The figure shows three views and two pictorial views of one solid part (mm, origin at its lowest corner). Answer the questions. A direction names the side the tool comes from. Coordinates: 2 decimals unless noted, no trailing zeros. Order: outer loops, then holes, each group sorted by start corner. A loop starts at its lowest first (then second) coordinate and runs counter-clockwise, first axis right, second up. Notation, with made-up numbers: (88.25, -30.75) -> (115.25, -30.75) arc R18 ccw to (115.25, -9.75) -> close; hole circle Ø3 at (2, 27). An arc over 180 degrees is marked (long way). Write item = value, one per line.
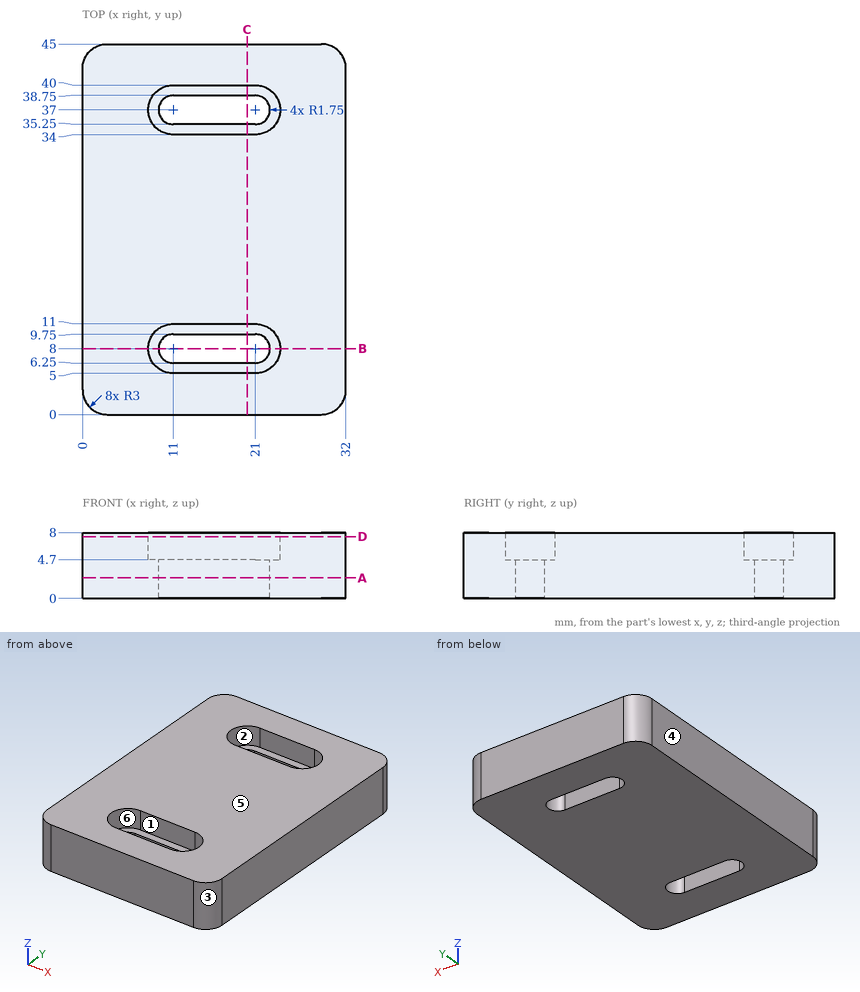
Q1. Section B-B, the plane y = 8 is taken. Give the vertices of the cut face in (x, z).
The answers:
outline = (0, 0) -> (9.25, 0) -> (9.25, 4.7) -> (8, 4.7) -> (8, 8) -> (0, 8) -> close; (22.75, 0) -> (32, 0) -> (32, 8) -> (24, 8) -> (24, 4.7) -> (22.75, 4.7) -> close
Q2. Find the intervals of material crossed by line 1 along Y through (x, z) = (13, 0.75); line 2 along X through (y, z) = (7, 6); line 3 along Z through (x, y) = (20, 10.5), in increasing order.
The answers:
line_1 = 0 to 6.25, 9.75 to 35.25, 38.75 to 45
line_2 = 0 to 8.17, 23.83 to 32
line_3 = 0 to 4.7
Q3. This flat-tipped pin is pushed along its axis until it touches: pin 1 Ø1.8 at (x, y) = (20, 36.5) entering from +Z. Where does it stop, or does it pass through?
The answers:
pin_1 = through
Q4. Section D-D, the plane z = 7.5 is taken. Give the vertices of the cut face in (x, y), plus the area to 3 significant figures.
The answers:
outline = (0, 3) arc R3 ccw to (3, 0) -> (29, 0) arc R3 ccw to (32, 3) -> (32, 42) arc R3 ccw to (29, 45) -> (3, 45) arc R3 ccw to (0, 42) -> close; hole (11, 5) -> (21, 5) arc R3 ccw to (21, 11) -> (11, 11) arc R3 ccw to start; hole (11, 34) -> (21, 34) arc R3 ccw to (21, 40) -> (11, 40) arc R3 ccw to start
area = 1,260 mm2
Q5. Section A-A, the plane z = 2.5 is taken. Give the vertices of the cut face in (x, y).
The answers:
outline = (0, 3) arc R3 ccw to (3, 0) -> (29, 0) arc R3 ccw to (32, 3) -> (32, 42) arc R3 ccw to (29, 45) -> (3, 45) arc R3 ccw to (0, 42) -> close; hole (11, 6.25) -> (21, 6.25) arc R1.75 ccw to (21, 9.75) -> (11, 9.75) arc R1.75 ccw to start; hole (11, 35.25) -> (21, 35.25) arc R1.75 ccw to (21, 38.75) -> (11, 38.75) arc R1.75 ccw to start
Q6. A tool of negligible diameter and unlimited length cuts with its end or side. For the marked faces 5 and 6, from which of +Z, -Z, +X, -X, +Y, -Y can it reach the whole face along a straight path? Write none if from no direction.
The answers:
face_5 = +Z, +X, -X, +Y, -Y
face_6 = +Z
Q7. Section C-C, the plane x = 20 is taken. Give the vertices of the cut face in (y, z), plus the area to 4 significant figures.
The answers:
outline = (0, 0) -> (6.25, 0) -> (6.25, 4.7) -> (5, 4.7) -> (5, 8) -> (0, 8) -> close; (9.75, 0) -> (35.25, 0) -> (35.25, 4.7) -> (34, 4.7) -> (34, 8) -> (11, 8) -> (11, 4.7) -> (9.75, 4.7) -> close; (38.75, 0) -> (45, 0) -> (45, 8) -> (40, 8) -> (40, 4.7) -> (38.75, 4.7) -> close
area = 287.5 mm2
Q8. The mould has two halves that part along X. Classify the marked faces 1, 2, 3 and 4: released by +X, released by -X, zero draft, split by the parting line, or undercut.
The answers:
face_1 = undercut
face_2 = undercut
face_3 = released by +X
face_4 = released by -X
